Answer from the drawing. Dimensions are ordinates in mm from the lowest x, y and z of the part. A direction names the side the tool comes from. Give positions to 0.01 mm unless a question says otherwise; leave off trailing zeros. Loops run counter-clockwise (first coordinate to the right, second up) from the corner with the lowest first, then second, coordinate; pieces in that order, holes last. Notation, with made-up numbers: (51, 1) - (66, 1) arc R20 ccw to (66, 31) - close; hole circle Ø10 at (21, 64). An arc over 180 degrees is marked (long way). One line per question, with ' | ' between items. Start each with the question number.
1. Section C-C (z = 95) is taken. Determine the outline of the cut face in (x, y), plus the area to 3 significant figures.
2. Section D-D (z = 27) is taken. Determine the outline of the cut face in (x, y).
3. Which of the six approach directions +Z, -Z, +X, -X, +Y, -Y give full straight-line access (tool end or side, diameter ignored) to the marked faces 1 and 2?
4. Find the intervals of material crossed by line 1 (X direction, y = 21, z = 95); line 2 (Y direction, x = 20, z = 15); line 3 (Z direction, x = 28, y = 13.5), in increasing order.
5. Section A-A (x = 23) is taken. Determine the outline of the cut face in (y, z).
6. Each of these flat-tipped pins is pushed along its axis until it touches: pin 1 (1 mm diameter, centred on x = 14.5, z = 111, fed in from +Y); pin 2 (6 mm diameter, centred on y = 46.5, z = 85, fed in from -X); pin 3 (6 mm diameter, centred on x = 75.5, y = 22, fed in from +Z). Where does it stop, or does it pass through?
7. Section B-B (y = 76) is taken. Determine the outline of the cut face in (x, z).
8. For a pull along X with two mould halves and no side action, classify the marked faces 3, 4, 5 and 6 as released by +X, released by -X, zero draft, split by the parting line, or undercut.
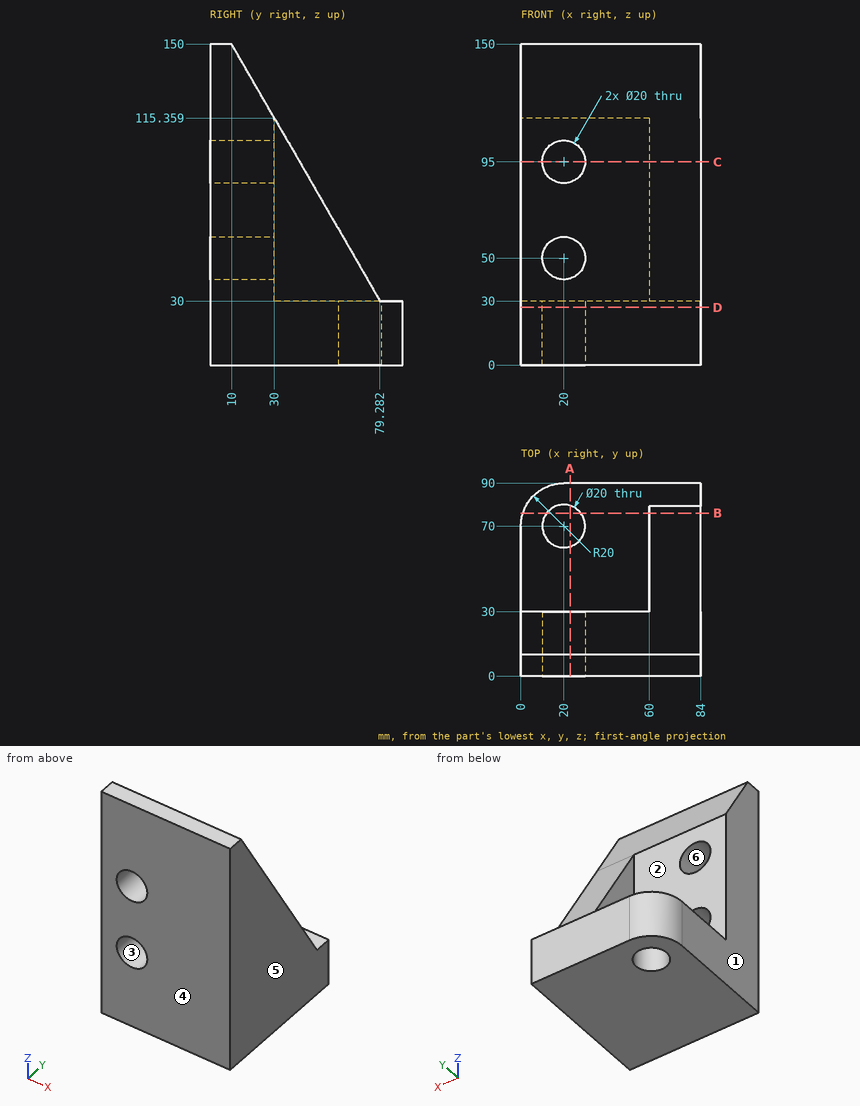
Conclusion:
1) outline: (0, 0) - (10, 0) - (10, 30) - (0, 30) - close; (30, 0) - (84, 0) - (84, 41.75) - (60, 41.75) - (60, 30) - (30, 30) - close | area: 2,200 mm²
2) outline: (0, 0) - (84, 0) - (84, 90) - (20, 90) arc R20 ccw to (0, 70) - close; hole circle Ø20 at (20, 70)
3) face 1: +Z, -Z, -X, +Y, -Y | face 2: +Z, -X, +Y
4) line 1: 0 to 10, 30 to 84 | line 2: 0 to 60, 80 to 90 | line 3: 0 to 44, 56 to 89, 101 to 143.94
5) outline: (0, 0) - (60.46, 0) - (60.46, 30) - (30, 30) - (30, 40.46) - (0, 40.46) - close; (0, 59.54) - (30, 59.54) - (30, 85.46) - (0, 85.46) - close; (0, 104.54) - (30, 104.54) - (30, 115.36) - (10, 150) - (0, 150) - close; (79.54, 0) - (90, 0) - (90, 30) - (79.54, 30) - close
6) pin 1: y = 30 | pin 2: x = 60 | pin 3: z = 134.41
7) outline: (0.92, 0) - (12, 0) - (12, 30) - (0.92, 30) - close; (28, 0) - (84, 0) - (84, 35.68) - (60, 35.68) - (60, 30) - (28, 30) - close
8) face 3: undercut | face 4: zero draft | face 5: released by +X | face 6: undercut
